Work out the finished part from the listing and answer in its coordinate system (mm). A direction names the side the tool comes from. Round coordinates to 2 decimals unless told otherwise and drop trailing zeros. Write each loop counter-clockwise with the first axis right and the second up, starting at its lowest first coordinate (ties: lowest second). Pieces come first, ordered by that corner, then holes.
from build123d import *

# Parameters (mm, degrees)
SKETCH_1_W                   = 30
SKETCH_1_H                   = 40
EXTRUDE_1_DEPTH              = 10
SKETCH_2_W                   = 40
SKETCH_2_H                   = 40
EXTRUDE_2_DEPTH              = 10
HOLE_WIZARD_M5_1_D           = 5.5
HOLE_WIZARD_M5_1_CBORE_D     = 10
HOLE_WIZARD_M5_1_CBORE_DEPTH = 5.4
CHAMFER_1_SIZE               = 0.5
CUT_EXTRUDE_1_DEPTH          = 49.989794856
CHAMFER_2_SIZE               = 0.5
CHAMFER_3_SIZE               = 0.5


with BuildPart() as part:
    # 草图1 → 凸台-拉伸1 (new body)
    with BuildSketch(Plane(origin=(0, 0, 0), x_dir=(1, 0, 0), z_dir=(0, 1, 0))):
        Rectangle(SKETCH_1_W, SKETCH_1_H)
    extrude(amount=EXTRUDE_1_DEPTH)

    # 草图2 → 凸台-拉伸2 (add)
    with BuildSketch(Plane.ZY.offset(15)):
        with Locations((0, 20)):
            Rectangle(SKETCH_2_W, SKETCH_2_H)
    extrude(amount=-EXTRUDE_2_DEPTH)

    # M5 六角凹头螺钉的柱形沉头孔1 (through all)
    with Locations(Plane(origin=(0, 10, 0), x_dir=(1, 0, 0), z_dir=(0, 1, 0))):
        with Locations((5, -12.5), (5, 12.5)):
            CounterBoreHole(HOLE_WIZARD_M5_1_D / 2, HOLE_WIZARD_M5_1_CBORE_D / 2, HOLE_WIZARD_M5_1_CBORE_DEPTH)

    # 倒角1
    chamfer_1_edges = [part.edges().sort_by_distance(p)[0] for p in [
        (15, 5, 20),
        (15, 5, -20),
    ]]
    chamfer(chamfer_1_edges, length=CHAMFER_1_SIZE)

    # 草图5 → 切除-拉伸1 (cut, through all)
    with BuildSketch(Plane(origin=(-5, 0, 0), x_dir=(0, 0, -1), z_dir=(1, 0, 0))):
        with BuildLine():
            Line((4.25, 30), (4.25, 20))
            ThreePointArc((4.25, 20), (0, 15.75), (-4.25, 20))
            Line((-4.25, 20), (-4.25, 30))
            ThreePointArc((-4.25, 30), (0, 34.25), (4.25, 30))
        make_face()
    extrude(amount=-CUT_EXTRUDE_1_DEPTH, mode=Mode.SUBTRACT)

    # 倒角2
    chamfer_2_edges = [part.edges().sort_by_distance(p)[0] for p in [
        (-10, 40, -20),
        (-10, 40, 20),
    ]]
    chamfer(chamfer_2_edges, length=CHAMFER_2_SIZE)

    # 倒角3
    chamfer_3_edges = [part.edges().sort_by_distance(p)[0] for p in [
        (4.75, 10, 20),
        (-5, 24.75, 20),
        (-0.25, 0, 20),
        (-15, 0, 0),
        (-0.25, 0, -20),
        (4.75, 10, -20),
        (15, 0, 0),
        (14.75, 0, 19.75),
        (14.75, 0, -19.75),
        (15, 10, 0),
        (14.75, 10, 19.75),
        (14.75, 10, -19.75),
        (-15, 19.75, 20),
        (-15, 40, 0),
        (-15, 19.75, -20),
        (-15, 39.75, -19.75),
        (-15, 39.75, 19.75),
        (-5, 40, 0),
        (-5, 24.75, -20),
        (-5, 39.75, -19.75),
        (-5, 39.75, 19.75),
    ]]
    chamfer(chamfer_3_edges, length=CHAMFER_3_SIZE)


solid = part.part
Q1. Find section B-B (z = 0). Determine the outline of the cut face in (x, y), plus the area to 3 significant figures.
Q2. A tool of negligible diameter and unlimited length cuts with its end or side. For faces 5 (the face through (-5, 25, -5)), 6 (the face through (-9.93, 15.75, -0.09)), 7 (the face through (0.005, 7.338, 12.28)), 8 (the face through (-15, 15, 0)), 9 (the face through (-10, 40, 0)), from which of +Z, -Z, +X, -X, +Y, -Y can it reach the whole face along a straight path? Write none if from no direction.
Q3. Find section C-C (y = 26). Determine the outline of the cut face in (x, z).
Q4. Find section D-D (x = -12.25). Determine the outline of the cut face in (y, z), plus the area to 3 significant figures.
Q5. Find the intervals of material crossed by L1, parallel to Z at x = 5, y = 5; L2, parallel to Z at x = 5, y = 3.2; L3, parallel to X at y = 2.4, z = 12.5, in increasing order.
Q6. Find section A-A (x = 5). Determine the outline of the cut face in (y, z), plus the area to 3 significant figures.
Q7. The mould has two halves that part along Z. Classify faces 1 (the face through (-7, 15, 20)), 2 (the face through (1.315, 7.338, -15.879)), 3 (the face through (15, 5, 0)), 4 (the face through (-7, 15, -20)): +Z half, -Z half, draft (parallel to the pull), parting line (faces both ways), or undercut.
Q8. Given pin 1 (12 mm diameter, centred on x = 4.5, y = 21.5, fed in from -Z); pin 2 (13 mm diameter, centred on x = 5, z = 12.5, fed in from +Y); pin 3 (12 mm diameter, centred on y = 13, z = -4, fed in from +X); pin 4 (9 mm diameter, centred on y = 24.5, z = -8.5, fed in from +X), each flat-ended and moving along its own axis, determine where each tip first touches the part or whether it passes through.
Report:
1. outline: (-15, 0.5) - (-14.5, 0) - (14.5, 0) - (15, 0.5) - (15, 9.5) - (14.5, 10) - (-5, 10) - (-5, 15.75) - (-15, 15.75) - close; (-15, 34.25) - (-5, 34.25) - (-5, 39.5) - (-5.5, 40) - (-14.5, 40) - (-15, 39.5) - close
1. area: 414 mm2
2. face 5: +Z, -Z, +X, +Y
2. face 6: +X, -X
2. face 7: +Y
2. face 8: +Z, -Z, -X, +Y, -Y
2. face 9: +Z, -Z, +X, -X, +Y
3. outline: (-15, -19.5) - (-14.5, -20) - (-5.5, -20) - (-5, -19.5) - (-5, -4.25) - (-15, -4.25) - close; (-15, 4.25) - (-5, 4.25) - (-5, 19.5) - (-5.5, 20) - (-14.5, 20) - (-15, 19.5) - close
4. outline: (0, -19.5) - (0.5, -20) - (39.5, -20) - (40, -19.5) - (40, 19.5) - (39.5, 20) - (0.5, 20) - (0, 19.5) - close; hole (20, -4.25) - (30, -4.25) arc R4.25 ccw to (30, 4.25) - (20, 4.25) arc R4.25 ccw to start
4. area: 1,460 mm2
5. L1: z = -20 to -17.5, -7.5 to 7.5, 17.5 to 20
5. L2: z = -20 to -15.25, -9.75 to 9.75, 15.25 to 20
5. L3: x = -15 to 2.25, 7.75 to 15
6. outline: (0, -19.5) - (0.5, -20) - (9.5, -20) - (10, -19.5) - (10, -17.5) - (4.6, -17.5) - (4.6, -15.25) - (0, -15.25) - close; (0, -9.75) - (4.6, -9.75) - (4.6, -7.5) - (10, -7.5) - (10, 7.5) - (4.6, 7.5) - (4.6, 9.75) - (0, 9.75) - close; (0, 15.25) - (4.6, 15.25) - (4.6, 17.5) - (10, 17.5) - (10, 19.5) - (9.5, 20) - (0.5, 20) - (0, 19.5) - close
6. area: 241 mm2
7. face 1: +Z half
7. face 2: undercut
7. face 3: draft
7. face 4: -Z half
8. pin 1: passes through
8. pin 2: stops at y = 10
8. pin 3: stops at x = 15
8. pin 4: stops at x = -5
